The model under review builds one solid part; all positions refer to its coordinate system, in mm. A direction names the side the tool comes from. Round coordinates to 2 decimals unless told otherwise and drop trailing zeros. Loops run counter-clockwise (first coordinate to the right, second up) from the corner with the lowest first, then second, coordinate; pieces in that order, holes last. Notation, with made-up numbers: M -33.75,0 L -9.75,0 A26 ccw -9.75,22 Z; hole C 5.25,48 d1. An arc over 180 degrees is marked long. Return JSON: item names as keys, results as strings. Group by question number.
Q1. To check wall thickness, follow line 1 along X through (y, z) = (10, 0.25); line 2 along Y through (x, z) = (-5.25, 3); line 3 along X through (y, z) = (33, -3). State the ranges of each line that lie inside material, in increasing order.
Q2. Consider section A-A (y = 33.5). State the section outline as (x, z) points (3 decimals), and give its area (3 significant figures).
Q3. Draft analysis for pull direction X (two halves, no side actions). For faces 1 (the face through (2, 29.5, 5)), 2 (the face through (-6.834, 30.634, -1.517)), 3 (the face through (-3.334, 37, 0)), state which applies: pulls with the +X half, pulls with the -X half, needs draft (parallel to the pull), parting line crosses it, or undercut.
Q4. Consider section B-B (z = 0). State the section outline as (x, y) points.
Q5. For faces 4 (the face through (2, 31.8, 6)), 5 (the face through (1.457, 15.05, 4.626)), 6 (the face through (0, 0, 0)), list the 3-axis set-ups (+Z, -Z, +X, -X, +Y, -Y) from which the entire face can be reached by the end or side of a thin tool; tool diameter is ignored.
Q6. Consider section C-C (y = 12). State the section outline as (x, z) points.
Q7. Clearance check with flat-ended pins moving along their axes: pin 1 Ø4 at (y, z) = (38.5, 0.5) entering from +X; pin 2 Ø1.5 at (x, y) = (0, 15) entering from +Z; pin 3 Ø1.2 at (y, z) = (35, -0.5) entering from -X. State where each tip first meets the part, or that it passes through.
from build123d import *

# Parameters (mm, degrees)
SHANK_SKETCH_9_7_R            = 4.85
SHANK_9_7X29_5_DEPTH          = 29.5
FLANGE_SKETCH_17_3_R          = 7
FLANGE_17_3X2_3_DEPTH         = 2.3
HEAD_SKETCH_12_R              = 6
HEAD_12X9_6_DEPTH             = 9.6
HEX_SOCKET_7_7X9_6_DEEP_DEPTH = 9.6
HEAD_TOP_CHAMFER_1X45_SIZE    = 1
SHANK_END_CHAMFER_1X45_SIZE   = 1


with BuildPart() as part:
    # Shank Sketch Ø9.7 → Shank Ø9.7x29.5 (new body)
    with BuildSketch(Plane(origin=(0, 0, 0), x_dir=(1, 0, 0), z_dir=(0, 1, 0))):
        with Locations(Location((0, 0, 0), (0, 0, 270))):
            Circle(SHANK_SKETCH_9_7_R)
    extrude(amount=SHANK_9_7X29_5_DEPTH)

    # Flange Sketch Ø17.3 → Flange Ø17.3x2.3 (add)
    with BuildSketch(Plane(origin=(0, 29.5, 0), x_dir=(1, 0, 0), z_dir=(0, 1, 0))):
        with Locations(Location((0, 0, 0), (0, 0, 270))):
            Circle(FLANGE_SKETCH_17_3_R)
    extrude(amount=FLANGE_17_3X2_3_DEPTH)

    # Head Sketch Ø12 → Head Ø12x9.6 (add)
    with BuildSketch(Plane(origin=(0, 31.8, 0), x_dir=(1, 0, 0), z_dir=(0, 1, 0))):
        with Locations(Location((0, 0, 0), (0, 0, 270))):
            Circle(HEAD_SKETCH_12_R)
    extrude(amount=HEAD_12X9_6_DEPTH)

    # Hex Socket Sketch 7.7 → Hex Socket 7.7x9.6 Deep (cut)
    with BuildSketch(Plane(origin=(0, 41.4, 0), x_dir=(1, 0, 0), z_dir=(0, 1, 0))):
        Polygon((0, 3.85), (-3.334197805, 1.925), (-3.334197805, -1.925), (0, -3.85), (3.334197805, -1.925), (3.334197805, 1.925), align=None)
    extrude(amount=-HEX_SOCKET_7_7X9_6_DEEP_DEPTH, mode=Mode.SUBTRACT)

    # Head Top Chamfer 1x45
    head_top_chamfer_1x45_edges = [part.edges().sort_by_distance(p)[0] for p in [
        (0, 41.4, -6),
    ]]
    chamfer(head_top_chamfer_1x45_edges, length=HEAD_TOP_CHAMFER_1X45_SIZE)

    # Shank End Chamfer 1x45
    shank_end_chamfer_1x45_edges = [part.edges().sort_by_distance(p)[0] for p in [
        (0, 0, -4.85),
    ]]
    chamfer(shank_end_chamfer_1x45_edges, length=SHANK_END_CHAMFER_1X45_SIZE)


solid = part.part
Values:
{
 "1": {"line 1": "x = -4.84 to 4.84", "line 2": "y = 29.5 to 31.8", "line 3": "x = -5.2 to -1.47, 1.47 to 5.2"},
 "2": {"outline": "C 0,0 d12; hole M -3.334,-1.925 L 0,-3.85 L 3.334,-1.925 L 3.334,1.925 L 0,3.85 L -3.334,1.925 Z", "area": "74.6 mm2"},
 "3": {"face 1": "needs draft", "face 2": "parting line crosses it", "face 3": "undercut"},
 "4": {"outline": "M -7,29.5 L -4.85,29.5 L -4.85,1 L -3.85,0 L 3.85,0 L 4.85,1 L 4.85,29.5 L 7,29.5 L 7,31.8 L 6,31.8 L 6,40.4 L 5,41.4 L 3.33,41.4 L 3.33,31.8 L -3.33,31.8 L -3.33,41.4 L -5,41.4 L -6,40.4 L -6,31.8 L -7,31.8 Z"},
 "5": {"face 4": "+Y", "face 5": "-Y", "face 6": "+Z, -Z, +X, -X, -Y"},
 "6": {"outline": "C 0,0 d9.7"},
 "7": {"pin 1": "stops at x = 6", "pin 2": "stops at z = 4.85", "pin 3": "stops at x = -6"}
}
